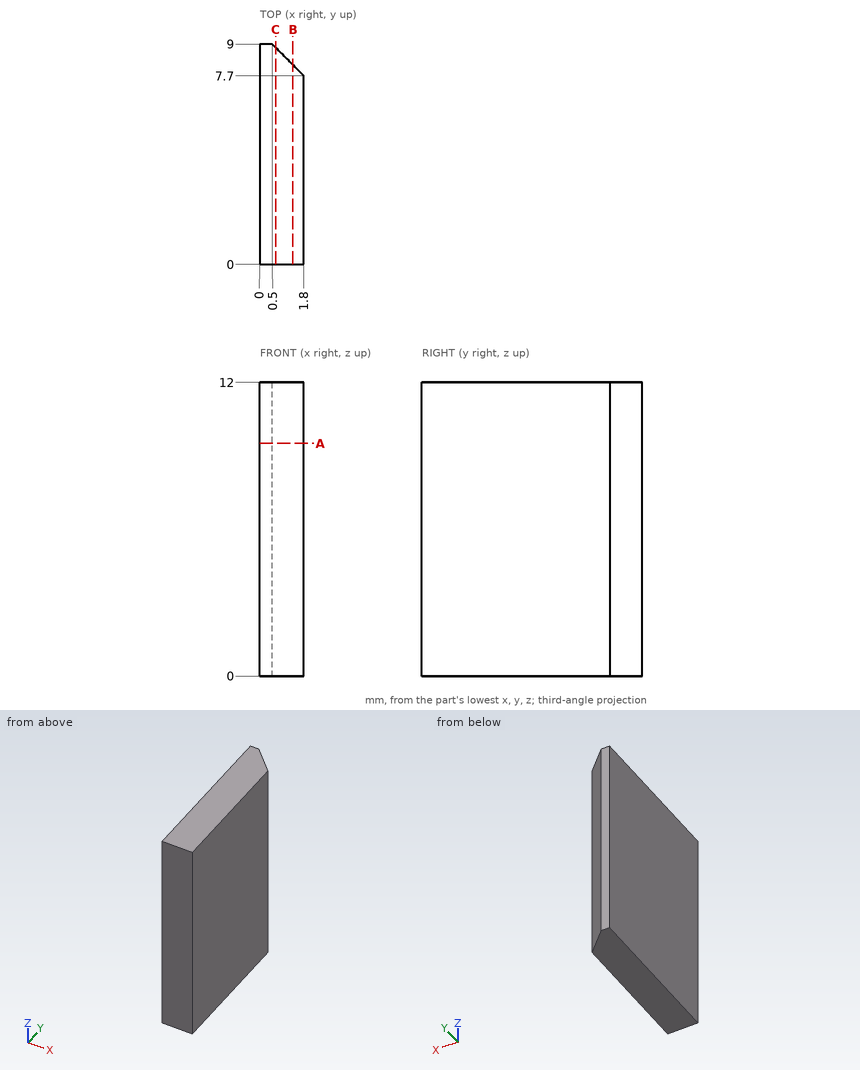
Source: three-view drawing plus pictorial views. Frame: mm from the lowest corner of the part. Coordinates: 2 decimals unless noted, no trailing zeros. Order: outer loops, then holes, each group sorted by start corner. A loop starts at its lowest first (then second) coordinate and runs counter-clockwise, first axis right, second up.
1) Section B-B (x = 1.35). Return loops of the section in (y, z).
Result sheet:
outline: (0, 0) - (8.15, 0) - (8.15, 12) - (0, 12) - close
2) Section A-A (z = 9.5). Return loops of the section in (x, y), then the cut area to 3 significant figures.
Result sheet:
outline: (0, 0) - (1.8, 0) - (1.8, 7.7) - (0.5, 9) - (0, 9) - close
area: 15.4 mm2
3) Ray query, probe 1 along Y at (x, z) = (1.05, 8.5); probe 2 along Y at (x, z) = (1.5, 3.75); probe 3 along X at (y, z) = (7.75, 8.5). Return the intervals inside material, ascending.
Result sheet:
probe 1: y = 0 to 8.45
probe 2: y = 0 to 8
probe 3: x = 0 to 1.75
4) First-contact query: P1, Ø5, axis at y = 7.5, z = 1.5, coming from the -X side. Flat tip, straight axial feed; report the tip coordinate or a pass-through.
Result sheet:
P1: stops at x = 0
5) Section C-C (x = 0.65). Return loops of the section in (y, z), then the cut area to 3 significant figures.
Result sheet:
outline: (0, 0) - (8.85, 0) - (8.85, 12) - (0, 12) - close
area: 106 mm2
